Part model, mm, in its own coordinate system. Give positions to 0.01 mm unless a question says otherwise; leave off trailing zeros. Loops run counter-clockwise (first coordinate to the right, second up) from the corner with the lowest first, then second, coordinate; pieces in that order, holes last. Notation, with made-up numbers: M 59,-24 L 112,-24 A32 cw 112,6 Z; hole C -7.75,18.5 d10. An arc over 180 degrees is marked long. Put each result on its own line as item: value. Start each with the question number.
```python
from build123d import *

# Parameters (mm, degrees)
SKETCH_1_R               = 122.5
SKETCH_1_R_2             = 65
EXTRUDE_1_DEPTH          = 3
SKETCH_2_W               = 5
SKETCH_2_H               = 9
CUT_EXTRUDE_1_DEPTH      = 5
PATTERN_CIRCULAR_1_COUNT = 8


with BuildPart() as part:
    # 草图1 → 凸台-拉伸1 (new body)
    with BuildSketch(Plane.XY):
        Circle(SKETCH_1_R)
        Circle(SKETCH_1_R_2, mode=Mode.SUBTRACT)
    extrude(amount=EXTRUDE_1_DEPTH)

    # 草图2 → 切除-拉伸1 (cut)
    with BuildSketch(Plane.XY.offset(3)):
        with Locations((0, 95)):
            Rectangle(SKETCH_2_W, SKETCH_2_H)
    cut_extrude_1 = extrude(amount=-CUT_EXTRUDE_1_DEPTH, mode=Mode.SUBTRACT)

    # 阵列(圆周)1: 切除-拉伸1 ×8 about axis
    pattern_circular_1_axis = Axis((0, 0, 0), (0, 0, 1))
    for i in range(1, PATTERN_CIRCULAR_1_COUNT):
        add(cut_extrude_1.rotate(pattern_circular_1_axis, i * 360 / PATTERN_CIRCULAR_1_COUNT), mode=Mode.SUBTRACT)


solid = part.part
```
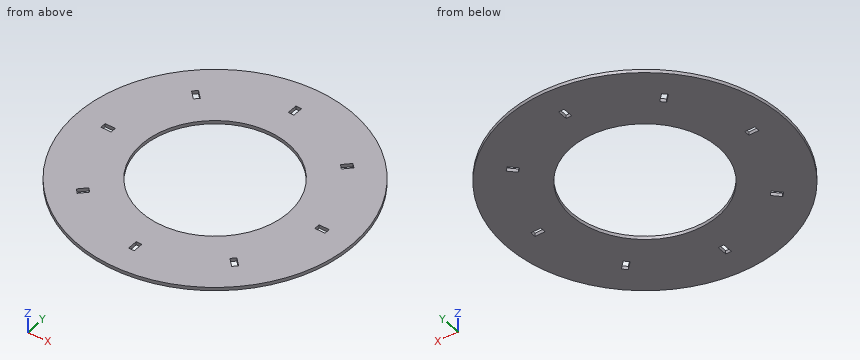
1) Wall check: L1, parallel to Y at x = 0, z = 1.55; L2, parallel to Y at x = 46, z = 1.9; L3, parallel to Y at x = 13.5, z = 0.55. Give the ranges that are in metal, low to high.
2) Band-saw the part on B-B on y = -93.5. Give the cut face in (x, z).
3) Band-saw the part on A-A on z = 0.65. State how many separate pieces and enclosed holes the cut face has, then the cut area to 3 significant figures.
4) Pin check, flat tips, straight feed: pin 1 Ø0.9 at (x, z) = (-97, 1.5) entering from -Y; pin 2 Ø1.5 at (y, z) = (1, 1) entering from +X; pin 3 Ø0.9 at (y, z) = (1, 1) entering from -X. Stop position of each tip, or through.
5) Band-saw the part on C-C on x = -49.5. Give the cut face in (y, z).
Evaluation:
1. L1: -122.5 to -99.5, -90.5 to -65, 65 to 90.5, 99.5 to 122.5
1. L2: -113.54 to -45.92, 45.92 to 113.54
1. L3: -121.75 to -63.58, 63.58 to 121.75
2. outline: M -79.15,0 L -2.5,0 L -2.5,3 L -79.15,3 Z; M 2.5,0 L 79.15,0 L 79.15,3 L 2.5,3 Z
3. separate pieces: 1
3. enclosed holes: 9
3. area: 33,500 mm2
4. pin 1: y = -75.39
4. pin 2: x = 122.5
4. pin 3: x = -122.5
5. outline: M -112.05,0 L -42.13,0 L -42.13,3 L -112.05,3 Z; M 42.13,0 L 112.05,0 L 112.05,3 L 42.13,3 Z
